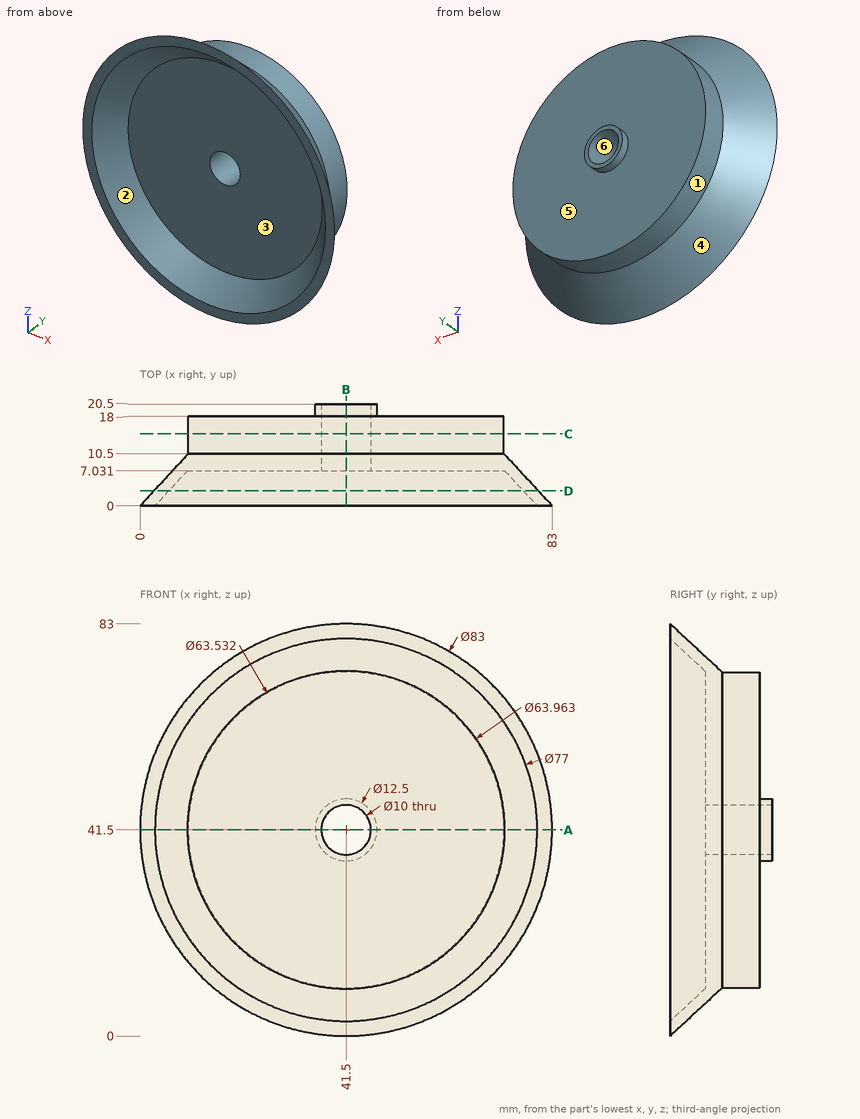
Study the drawing (mm; zero at the part's minimum x, y, z) and answer. A direction names the side the tool comes from. Give positions to 0.01 mm unless a question says otherwise; leave off trailing zeros. Write each loop counter-clockwise with the first axis right and the second up, starting at its lowest first coordinate (ties: lowest second). Pieces come first, ordered by that corner, then holes. Notation, with made-up numbers: (47, 80) -> (95, 80) arc R12 cw to (95, 91) -> close; hole circle Ø6 at (51.25, 51). An arc over 180 degrees is marked (long way). Answer as a JSON object with one key per item and string values. Group by question number.
1) Find section C-C (y = 14.5). Write down the section's boundary in (x, z), and give its area (3 significant figures).
2) The mould has two halves that part along Z. Classify the marked faces 3, 4, 5 and 6: +Z half, -Z half, draft (parallel to the pull), parting line (faces both ways), or undercut.
3) Find section D-D (y = 3). Write down the section's boundary in (x, z).
4) A tool of negligible diameter and unlimited length cuts with its end or side. For the marked faces 1 and 2, from which of +Z, -Z, +X, -X, +Y, -Y can it reach the whole face along a straight path? Write none if from no direction.
5) Consider L1, parallel to Y at x = 40.5, z = 13.5; L2, parallel to X at y = 17.5, z = 41.5; L3, parallel to Z at x = 48, y = 2.75 (1 decimal). Determine where each line is inside the solid, lowest interval first. Write a range as from..to.
6) Find section A-A (z = 41.5). Write down the section's boundary in (x, y), and give its area (3 significant figures).
7) Find section B-B (x = 41.5). Write down the section's boundary in (y, z), and give its area (3 significant figures).
8) Each of these flat-tipped pins is pushed along its axis until it touches: P1, Ø12, axis at x = 59.5, y = 12.5, coming from the -Z side (1 decimal); P2, Ø8, axis at y = 8, z = 55.5, coming from the -X side; P3, Ø4, axis at x = 13.5, y = 14.5, coming from the -Z side; P4, Ø9, axis at x = 41.5, z = 41.5, coming from the -Y side. Where does it stop, or does it pass through?
Values follow:
{
 "1": {"outline": "circle Ø63.53 at (41.5, 41.5); hole circle Ø10 at (41.5, 41.5)", "area": "3,090 mm2"},
 "2": {"face 3": "undercut", "face 4": "parting line", "face 5": "draft", "face 6": "undercut"},
 "3": {"outline": "circle Ø77.44 at (41.5, 41.5); hole circle Ø71.44 at (41.5, 41.5)"},
 "4": {"face 1": "+Y", "face 2": "-Y"},
 "5": {"L1": "y = 7.03..18", "L2": "x = 9.73..36.5, 46.5..73.27", "L3": "z = 3.1..6.1, 76.9..79.9"},
 "6": {"outline": "(0, 0) -> (3, 0) -> (9.52, 7.03) -> (36.5, 7.03) -> (36.5, 20.5) -> (35.25, 20.5) -> (35.25, 18) -> (9.73, 18) -> (9.73, 10.5) -> close; (46.5, 7.03) -> (73.48, 7.03) -> (80, 0) -> (83, 0) -> (73.27, 10.5) -> (73.27, 18) -> (47.75, 18) -> (47.75, 20.5) -> (46.5, 20.5) -> close", "area": "647 mm2"},
 "7": {"outline": "(0, 0) -> (10.5, 9.73) -> (18, 9.73) -> (18, 35.25) -> (20.5, 35.25) -> (20.5, 36.5) -> (7.03, 36.5) -> (7.03, 9.52) -> (0, 3) -> close; (0, 80) -> (7.03, 73.48) -> (7.03, 46.5) -> (20.5, 46.5) -> (20.5, 47.75) -> (18, 47.75) -> (18, 73.27) -> (10.5, 73.27) -> (0, 83) -> close", "area": "647 mm2"},
 "8": {"P1": "stops at z = 10.2", "P2": "stops at x = 6.12", "P3": "stops at z = 23.25", "P4": "passes through"}
}
